Source: CAD feature listing. Evaluate the final solid. Frame: model axes, mm. Face numbers are marked on the shaded views. A direction names the side the tool comes from. Coordinates: 2 decimals unless noted, no trailing zeros. One line per question, with ' | ' between items. Start each with the question number.
Q1. Cut plane A-A, the plane y = 0. Give the number of separate pieces and of enclosed holes in the cut face, plus the area to 3 significant figures.
Q2. Access query for the marked faces 4, 5, 6, 7 and 8. Directions: +Z, -Z, +X, -X, +Y, -Y. A direction counts if a zero-diameter tool reaches every point of the face in a straight line with its end or side. Return the directions, or none.
Q3. Line query: line 1 (Y direction, x = 26, z = 0); line 2 (X direction, y = -37, z = -73); line 3 (Y direction, x = 24, z = -64.5). Output: solid intervals per line, ascending.
Q4. Draft query along Z for the marked faces 1, 2 and 3. Return one class per face: +Z half, -Z half, draft (parallel to the pull), parting line (faces both ways), or undercut.
Q5. Contact query for flat-ended pins moving along their axis: P1, Ø25, axis at y = 1.5, z = 0.5, coming from the -X side; P2, Ø5, axis at y = 66, z = 57, coming from the +X side; P3, Ø3.5, axis at x = 17.5, z = -14.5, coming from the +Y side; P4, Ø21.5, axis at y = 0, z = 62.5, coming from the +X side. Output: stop coordinate, or through.
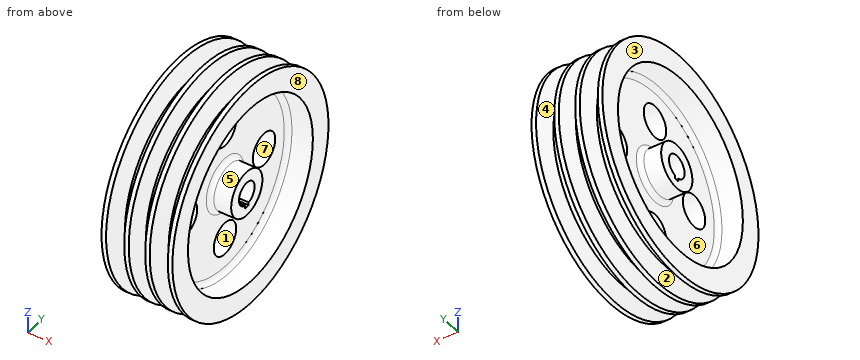
```python
from build123d import *

# Parameters (mm, degrees)
EDGE_FILLET_R5_A_R           = 5
EDGE_FILLET_R5_B_R           = 5
EDGE_FILLET_R5_C_R           = 5
KEYWAY_6X6_DEPTH             = 80
LIGHTENING_HOLES_SKETCH_R    = 18
LIGHTENING_HOLES_4X_36_DEPTH = 45


with BuildPart() as part:
    # Pulley Profile Sketch → Pulley Body Revolve (revolve)
    with BuildSketch(Plane.XY, mode=Mode.PRIVATE) as pulley_body_revolve_sk:
        Polygon((-35, 12.5), (35, 12.5), (35, 25), (11, 25), (11, 100), (39, 100), (39, 125), (34, 125), (27.448535783, 107), (22.448535783, 107), (14.051464217, 125), (9.051464217, 125), (2.5, 107), (-2.5, 107), (-9.051464217, 125), (-14.051464217, 125), (-20.602928434, 107), (-25.602928434, 107), (-34, 125), (-39, 125), (-39, 100), (-11, 100), (-11, 25), (-35, 25), align=None)
    revolve(pulley_body_revolve_sk.sketch.rotate(Axis((-52.075788227, 0, 0), (1, 0, 0)), 90), axis=Axis((-52.075788227, 0, 0), (1, 0, 0)))

    # Edge Fillet R5 A
    edge_fillet_r5_a_edges = [part.edges().sort_by_distance(p)[0] for p in [
        (11, 0, -100),
    ]]
    fillet(edge_fillet_r5_a_edges, radius=EDGE_FILLET_R5_A_R)

    # Edge Fillet R5 B
    edge_fillet_r5_b_edges = [part.edges().sort_by_distance(p)[0] for p in [
        (11, 0, -25),
    ]]
    fillet(edge_fillet_r5_b_edges, radius=EDGE_FILLET_R5_B_R)

    # Edge Fillet R5 C
    edge_fillet_r5_c_edges = [part.edges().sort_by_distance(p)[0] for p in [
        (-11, 0, -25),
        (-11, 0, -100),
    ]]
    fillet(edge_fillet_r5_c_edges, radius=EDGE_FILLET_R5_C_R)

    # Keyway Sketch → Keyway 6x6 (cut)
    with BuildSketch(Plane(origin=(35, 0, 0), x_dir=(0, 0, -1), z_dir=(1, 0, 0))):
        with BuildLine():
            Line((12.1346611, 3), (15.5, 3))
            Line((15.5, 3), (15.5, -3))
            Line((15.5, -3), (12.1346611, -3))
            ThreePointArc((12.1346611, -3), (12.5, 0), (12.1346611, 3))
        make_face()
    extrude(amount=-KEYWAY_6X6_DEPTH, mode=Mode.SUBTRACT)

    # Lightening Holes Sketch → Lightening Holes 4xØ36 (cut, symmetric)
    with BuildSketch(Plane(origin=(11, 0, 0), x_dir=(0, 0, -1), z_dir=(1, 0, 0))):
        with Locations((0, 62.5)):
            Circle(LIGHTENING_HOLES_SKETCH_R)
        with Locations((62.5, 0)):
            Circle(LIGHTENING_HOLES_SKETCH_R)
        with Locations((0, -62.5)):
            Circle(LIGHTENING_HOLES_SKETCH_R)
        with Locations((-62.5, 0)):
            Circle(LIGHTENING_HOLES_SKETCH_R)
    extrude(amount=LIGHTENING_HOLES_4X_36_DEPTH, both=True, mode=Mode.SUBTRACT)


solid = part.part
```
Reply:
1) separate pieces: 4 | enclosed holes: 0 | area: 5,880 mm^2
2) face 4: none | face 5: +X | face 6: -X | face 7: +X, -X | face 8: +Z, -Z, +X, +Y, -Y
3) line 1: y = -107 to -100, -25 to -12.5, 12.5 to 25, 100 to 107 | line 2: x = -11 to 11 | line 3: y = -85.37 to -76.42, 76.42 to 85.37
4) face 1: undercut | face 2: parting line | face 3: draft
5) P1: stops at x = -35 | P2: stops at x = 11 | P3: stops at y = 120.5 | P4: passes through
